Geometry: final body of the model. Coordinates: model frame, mm. Face numbers are marked on the shaded views. Round coordinates to 2 decimals unless told otherwise and drop trailing zeros. Order: outer loops, then holes, each group sorted by start corner. A loop starts at its lowest first (then second) coordinate and runs counter-clockwise, first axis right, second up. Notation, with made-up numbers: (-34, 70.5) -> (16, 70.5) arc R15 cw to (16, 91.5) -> close; hole circle Ø11 at (62, 58.5). An arc over 180 degrees is marked (long way). Put each result on its own line as item: value.
```python
from build123d import *

# Parameters (mm, degrees)
SKETCH_1_W                = 900
SKETCH_1_H                = 635
EXTRUDE_1_DEPTH           = 5
SKETCH_2_W                = 25
SKETCH_2_H                = 635
EXTRUDE_2_DEPTH           = 20
SKETCH_4_W                = 850
SKETCH_4_H                = 25
EXTRUDE_3_DEPTH           = 20
SKETCH_5_W                = 25
SKETCH_5_H                = 585
EXTRUDE_4_DEPTH           = 20
SKETCH_6_W                = 850
SKETCH_6_H                = 25
EXTRUDE_5_DEPTH           = 20
SKETCH_7_W                = 526
SKETCH_7_H                = 10
EXTRUDE_6_DEPTH           = 35
HOLE_WIZARD_1_D           = 11
HOLE_WIZARD_1_CBORE_D     = 17
HOLE_WIZARD_1_CBORE_DEPTH = 6.85
HOLE_WIZARD_2_D           = 5.5
HOLE_WIZARD_2_CBORE_D     = 9
HOLE_WIZARD_2_CBORE_DEPTH = 15


with BuildPart() as part:
    # 草图1 → 拉伸1 (new body)
    with BuildSketch(Plane(origin=(0, 0, 0), x_dir=(0, 0, -1), z_dir=(1, 0, 0))):
        with Locations((450, 317.5)):
            Rectangle(SKETCH_1_W, SKETCH_1_H)
    extrude(amount=EXTRUDE_1_DEPTH)

    # 草图2 → 拉伸2 (add)
    with BuildSketch(Plane(origin=(5, 0, 0), x_dir=(0, 0, -1), z_dir=(1, 0, 0))):
        with Locations((12.5, 317.5)):
            Rectangle(SKETCH_2_W, SKETCH_2_H)
        with Locations((887.5, 317.5)):
            Rectangle(SKETCH_2_W, SKETCH_2_H)
    extrude(amount=EXTRUDE_2_DEPTH)

    # 草图4 → 拉伸3 (add)
    with BuildSketch(Plane(origin=(5, 0, 0), x_dir=(0, 0, -1), z_dir=(1, 0, 0))):
        with Locations((450, 622.5)):
            Rectangle(SKETCH_4_W, SKETCH_4_H)
        with Locations((450, 12.5)):
            Rectangle(SKETCH_4_W, SKETCH_4_H)
    extrude(amount=EXTRUDE_3_DEPTH)

    # 草图5 → 拉伸4 (add)
    with BuildSketch(Plane(origin=(5, 0, 0), x_dir=(0, 0, -1), z_dir=(1, 0, 0))):
        with Locations((307.5, 317.5)):
            Rectangle(SKETCH_5_W, SKETCH_5_H)
        with Locations((592.5, 317.5)):
            Rectangle(SKETCH_5_W, SKETCH_5_H)
    extrude(amount=EXTRUDE_4_DEPTH)

    # 草图6 → 拉伸5 (add)
    with BuildSketch(Plane(origin=(5, 0, 0), x_dir=(0, 0, -1), z_dir=(1, 0, 0))):
        with Locations((450, 317.5)):
            Rectangle(SKETCH_6_W, SKETCH_6_H)
    extrude(amount=EXTRUDE_5_DEPTH)

    # 草图7 → 拉伸6 (add)
    with BuildSketch(Plane(origin=(25, 0, 0), x_dir=(0, 0, -1), z_dir=(1, 0, 0))):
        with Locations((450, 5)):
            Rectangle(SKETCH_7_W, SKETCH_7_H)
    extrude(amount=EXTRUDE_6_DEPTH)

    # 孔1 (through all)
    with Locations(Plane(origin=(42.5, 10, -675), x_dir=(0, 0, 1), z_dir=(0, 1, 0))):
        with Locations((0, 0), (150, 0), (300, 0), (450, 0)):
            CounterBoreHole(HOLE_WIZARD_1_D / 2, HOLE_WIZARD_1_CBORE_D / 2, HOLE_WIZARD_1_CBORE_DEPTH)

    # 孔2 (through all)
    with Locations(Plane(origin=(25, 617.5, -12.5), x_dir=(0, 0, 1), z_dir=(1, 0, 0))):
        with Locations((0, 0), (0, 120), (0, 240), (0, 360), (0, 480), (0, 600)):
            hole_wizard_2 = CounterBoreHole(HOLE_WIZARD_2_D / 2, HOLE_WIZARD_2_CBORE_D / 2, HOLE_WIZARD_2_CBORE_DEPTH)

    # 镜向1: 孔2 across plane
    add(hole_wizard_2.mirror(Plane.XY.offset(-450)), mode=Mode.SUBTRACT)


solid = part.part
```
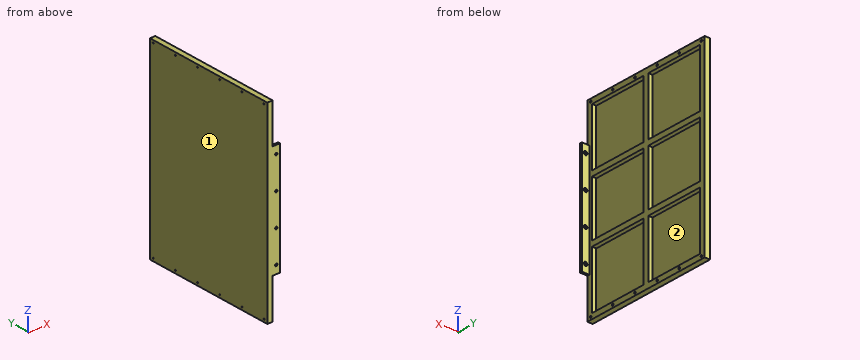
1. Draft query along Z for the marked faces 1 and 2. Return one class per face: +Z half, -Z half, draft (parallel to the pull), parting line (faces both ways), or undercut.
Ans:
face 1: draft
face 2: undercut
2. Material intervals for probe 1 along Z at (x, y) = (11.5, 359); probe 2 along Y at (x, z) = (14.5, -119.5); probe 3 along Z at (x, y) = (4, 497.5), sorted ascending.
Ans:
probe 1: -900 to -875, -605 to -580, -320 to -295, -25 to 0
probe 2: 0 to 25, 305 to 330, 610 to 635
probe 3: -900 to -890.25, -884.75 to -15.25, -9.75 to 0
3. Contact query for flat-ended pins moving along their axis: P1, Ø2, axis at y = 273, z = -726, coming from the +X side; P2, Ø14.5, axis at y = 257.5, z = -12.5, coming from the +X side; P3, Ø10, axis at x = 42.5, z = -525, coming from the +Y side; P4, Ø8, axis at y = 377.5, z = -887.5, coming from the +X side. Output: stop coordinate, or through.
Ans:
P1: x = 5
P2: x = 25
P3: through
P4: x = 10
4. Cut plane B-B on y = 72.5. Return loops of the section in (x, z), and give its area (3 significant figures).
Ans:
outline: (0, -900) -> (25, -900) -> (25, -875) -> (5, -875) -> (5, -605) -> (25, -605) -> (25, -580) -> (5, -580) -> (5, -320) -> (25, -320) -> (25, -295) -> (5, -295) -> (5, -25) -> (25, -25) -> (25, 0) -> (0, 0) -> close
area: 6,500 mm²
5. Cut plane A-A on z = -419. Return loops of the section in (x, y), and give its area (4 significant figures).
Ans:
outline: (0, 0) -> (60, 0) -> (60, 10) -> (25, 10) -> (25, 25) -> (5, 25) -> (5, 305) -> (25, 305) -> (25, 330) -> (5, 330) -> (5, 610) -> (25, 610) -> (25, 635) -> (0, 635) -> close
area: 5,025 mm²
6. Cut plane C-C on z = -135.5. Return loops of the section in (x, y), and give its area (4 significant figures).
Ans:
outline: (0, 0) -> (25, 0) -> (25, 25) -> (5, 25) -> (5, 305) -> (25, 305) -> (25, 330) -> (5, 330) -> (5, 610) -> (25, 610) -> (25, 635) -> (0, 635) -> close
area: 4,675 mm²
